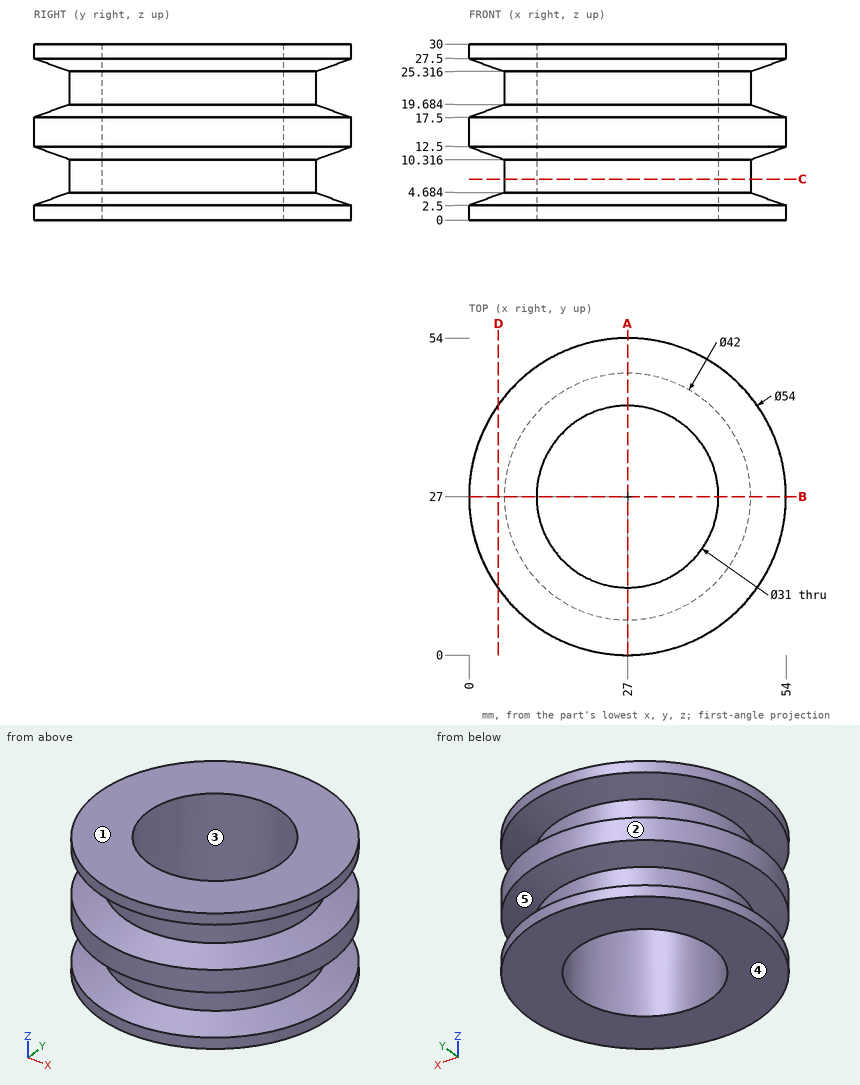
Could you check a few things on this drawing? It's one solid part, dimensions in mm from its lowest x, y, z. A direction names the side the tool comes from. Coordinates: 2 decimals unless noted, no trailing zeros. Order: outer loops, then holes, each group sorted by start corner. A loop starts at its lowest first (then second) coordinate and runs counter-clockwise, first axis right, second up.
1. I'm going to push flat-ended pins straight in: pin 1 (10 mm diameter, centred on y = 10.5, z = 15, fed in from -X); pin 2 (2 mm diameter, centred on x = 42.5, y = 17, fed in from -Z); pin 3 (8 mm diameter, centred on x = 11, z = 14.5, fed in from +Y); pin 4 (10 mm diameter, centred on x = 6, z = 23.5, fed in from +Y) (1 decimal). Where does each tip first touch, or does it pass through?
2. If we section it at D-D (x = 5): Give the number of separate pieces and of enclosed holes in the cut face, then the cut area to 3 significant figures.
3. If we section it at A-A (x = 27): Please give me the cut outline in (y, z), then the cut area to 3 significant figures.
4. I need wall thicknesses on line 1 (Y direction, x = 27, z = 6.5); line 2 (Z direction, x = 48.5, y = 31); line 3 (Z direction, x = 48, y = 42.5). Which ranges of each line are inside material? Lowest first, please.
5. If we section it at C-C (z = 7): Please give me the cut outline in (x, y), then the cut area to 3 significant figures.
6. For the marked faces 4 and 5, which set-ups out of +Z, -Z, +X, -X, +Y, -Y let a thin tool reach every point of the face, with its end or its side?
7. Thinking about a two-plate mould opening in X: for the marked faces 1, 2 and 3, which applies, +X half, -X half, draft (parallel to the pull), parting line (faces both ways), or undercut?
Entries:
1. pin 1: stops at x = 2.57
1. pin 2: stops at z = 0
1. pin 3: stops at y = 51.19
1. pin 4: stops at y = 47.1
2. separate pieces: 3
2. enclosed holes: 0
2. area: 462 mm2
3. outline: (0, 0) - (11.5, 0) - (11.5, 30) - (0, 30) - (0, 27.5) - (6, 25.32) - (6, 19.68) - (0, 17.5) - (0, 12.5) - (6, 10.32) - (6, 4.68) - (0, 2.5) - close; (42.5, 0) - (54, 0) - (54, 2.5) - (48, 4.68) - (48, 10.32) - (54, 12.5) - (54, 17.5) - (48, 19.68) - (48, 25.32) - (54, 27.5) - (54, 30) - (42.5, 30) - close
3. area: 502 mm2
4. line 1: y = 6 to 11.5, 42.5 to 48
4. line 2: z = 0 to 4.37, 10.63 to 19.37, 25.63 to 30
4. line 3: z = 0 to 2.83, 12.17 to 17.83, 27.17 to 30
5. outline: circle Ø42 at (27, 27); hole circle Ø31 at (27, 27)
5. area: 631 mm2
6. face 4: -Z, +X, -X, +Y, -Y
6. face 5: none
7. face 1: draft
7. face 2: parting line
7. face 3: undercut
